The listing builds one solid part. Answer for the finished solid, in the listing's coordinates (mm). Face numbers are marked on the shaded views. A direction names the side the tool comes from. Coordinates: 2 decimals unless noted, no trailing zeros. Loops run counter-clockwise (first coordinate to the right, second up) from the corner with the lowest first, then second, coordinate; pieces in that order, holes last. Notation, with made-up numbers: (67, -7) - (82, -7) arc R20 cw to (82, 18) - close; hole circle Ø7 at (73, 69). An arc over 180 degrees is marked (long way). Write each question's results on one line, items separated by ' | '. Start each with the question number.
(1) Find section A-A on z = -37.5. Determine the outline of the cut face in (x, y).
(2) Given pin 1 Ø6 at (x, z) = (44, -5) entering from +Y; pin 2 Ø10 at (x, y) = (135.5, 79) entering from +Z; pin 3 Ø12 at (x, z) = (49.5, -67) entering from +Y; pin 4 Ø10 at (x, z) = (126, -11.5) entering from -Y, each flat-ended and moving along its own axis, determine where each tip first touches the part or whether it passes through.
(3) For the marked faces 4, 5, 6 and 7, determine the directions among +Z, -Z, +X, -X, +Y, -Y from which every point of the face is accessible in a straight line to the end or side of a thin tool.
(4) Find section C-C on y = 20. Determine the outline of the cut face in (x, z), then the cut area to 4 significant figures.
(5) Find section B-B on x = -175. Determine the outline of the cut face in (y, z).
(6) Find section D-D on z = -17.5. Determine the outline of the cut face in (x, y), then the cut area to 3 significant figures.
(7) Determine the mould class of the marked faces 1, 2 and 3 for opening direction X: released by +X, released by -X, zero draft, split by the parting line, or undercut.
(8) Consider line 1 (X direction, y = 36, z = -46.5); line 2 (Y direction, x = 0, z = -19); line 3 (Y direction, x = 0, z = -1.9). Determine where each line is inside the solid, lowest interval first. Write a range as from..to.
from build123d import *

# Parameters (mm, degrees)
SUPPORT_BODY_DEPTH           = 75
RIB_FRONT_DEPTH              = 12.5
RIB_START                    = -12.5
RIB_BACK_DEPTH               = 12.5
MOUNTING_HOLES_SKETCH_R      = 12.5
MOUNTING_HOLES_2X_25_DEPTH   = 108.5
FLANGE_FILLET_R12_5_A_R      = 12.5
FLANGE_FILLET_R12_5_B_R      = 12.5
FLANGE_FILLET_R12_5_C_R      = 12.5
FLANGE_FILLET_R12_5_D_R      = 12.5
COUNTERBORE_FRONT_SKETCH_R   = 25
COUNTERBORE_FRONT_50X5_DEPTH = 5
SHAFT_BORE_SKETCH_R          = 20
SHAFT_BORE_40_DEPTH          = 98
COUNTERBORE_START            = -5
COUNTERBORE_BACK_SKETCH_R    = 25
COUNTERBORE_BACK_50X5_DEPTH  = 5


with BuildPart() as part:
    # Support Profile Sketch → Support Body (new body)
    with BuildSketch(Plane.XY):
        with BuildLine():
            Line((33.541019662, 30), (62.5, 30))
            Line((62.5, 30), (137.5, 105))
            Line((137.5, 105), (212.5, 105))
            Line((212.5, 105), (212.5, 90))
            Line((212.5, 90), (137.5, 90))
            Line((137.5, 90), (82.5, 30))
            Line((82.5, 30), (82.5, 0))
            Line((82.5, 0), (82.5, -30))
            Line((82.5, -30), (-82.5, -30))
            Line((-82.5, -30), (-82.5, 30))
            Line((-82.5, 30), (-137.5, 90))
            Line((-137.5, 90), (-212.5, 90))
            Line((-212.5, 90), (-212.5, 105))
            Line((-212.5, 105), (-137.5, 105))
            Line((-137.5, 105), (-62.5, 30))
            Line((-62.5, 30), (-33.541019662, 30))
            ThreePointArc((-33.541019662, 30), (0, 55), (33.541019662, 30))
        make_face()
    extrude(amount=-SUPPORT_BODY_DEPTH)

    # Rib Front Sketch → Rib Front (add)
    with BuildSketch(Plane.XY.offset(-12.5)):
        with BuildLine():
            Line((137.5, 105), (0, 55))
            ThreePointArc((0, 55), (20.916500663, 48.062430401), (33.541019662, 30))
            Line((33.541019662, 30), (62.5, 30))
            Line((62.5, 30), (137.5, 105))
        make_face()
        with BuildLine():
            ThreePointArc((-33.541019662, 30), (-20.916500663, 48.062430401), (0, 55))
            Line((0, 55), (-137.5, 105))
            Line((-137.5, 105), (-62.5, 30))
            Line((-62.5, 30), (-33.541019662, 30))
        make_face()
    extrude(amount=-RIB_FRONT_DEPTH)

    # Rib Back Sketch → Rib Back (add)
    with BuildSketch(Plane(origin=(0, 0, -62.5), x_dir=(-1, 0, 0), z_dir=(0, 0, -1)).offset(RIB_START)):
        with BuildLine():
            Line((137.5, 105), (0, 55))
            ThreePointArc((0, 55), (20.916500663, 48.062430401), (33.541019662, 30))
            Line((33.541019662, 30), (62.5, 30))
            Line((62.5, 30), (137.5, 105))
        make_face()
        with BuildLine():
            Line((0, 55), (-137.5, 105))
            Line((-137.5, 105), (-62.5, 30))
            Line((-62.5, 30), (-33.541019662, 30))
            ThreePointArc((-33.541019662, 30), (-20.916500663, 48.062430401), (0, 55))
        make_face()
    extrude(amount=RIB_BACK_DEPTH)

    # Mounting Holes Sketch → Mounting Holes 2xØ25 (cut)
    with BuildSketch(Plane(origin=(0, 105, 0), x_dir=(1, 0, 0), z_dir=(0, 1, 0))):
        with Locations(Location((175, 37.5, 0), (0, 0, 270))):
            Circle(MOUNTING_HOLES_SKETCH_R)
        with Locations(Location((-175, 37.5, 0), (0, 0, 90))):
            Circle(MOUNTING_HOLES_SKETCH_R)
    extrude(amount=-MOUNTING_HOLES_2X_25_DEPTH, mode=Mode.SUBTRACT)

    # Flange Fillet R12.5 A
    flange_fillet_r12_5_a_edges = [part.edges().sort_by_distance(p)[0] for p in [
        (212.5, 97.5, 0),
    ]]
    fillet(flange_fillet_r12_5_a_edges, radius=FLANGE_FILLET_R12_5_A_R)

    # Flange Fillet R12.5 B
    flange_fillet_r12_5_b_edges = [part.edges().sort_by_distance(p)[0] for p in [
        (212.5, 97.5, -75),
    ]]
    fillet(flange_fillet_r12_5_b_edges, radius=FLANGE_FILLET_R12_5_B_R)

    # Flange Fillet R12.5 C
    flange_fillet_r12_5_c_edges = [part.edges().sort_by_distance(p)[0] for p in [
        (-212.5, 97.5, -75),
    ]]
    fillet(flange_fillet_r12_5_c_edges, radius=FLANGE_FILLET_R12_5_C_R)

    # Flange Fillet R12.5 D
    flange_fillet_r12_5_d_edges = [part.edges().sort_by_distance(p)[0] for p in [
        (-212.5, 97.5, 0),
    ]]
    fillet(flange_fillet_r12_5_d_edges, radius=FLANGE_FILLET_R12_5_D_R)

    # Counterbore Front Sketch → Counterbore Front Ø50x5 (cut)
    with BuildSketch(Plane.XY):
        with Locations((0, 20)):
            Circle(COUNTERBORE_FRONT_SKETCH_R)
    extrude(amount=-COUNTERBORE_FRONT_50X5_DEPTH, mode=Mode.SUBTRACT)

    # Shaft Bore Sketch → Shaft Bore Ø40 (cut)
    with BuildSketch(Plane.XY.offset(-5)):
        with Locations((0, 20)):
            Circle(SHAFT_BORE_SKETCH_R)
    extrude(amount=-SHAFT_BORE_40_DEPTH, mode=Mode.SUBTRACT)

    # Counterbore Back Sketch → Counterbore Back Ø50x5 (cut)
    with BuildSketch(Plane(origin=(0, 0, -75), x_dir=(-1, 0, 0), z_dir=(0, 0, -1)).offset(COUNTERBORE_START)):
        with Locations(Location((0, 20, 0), (0, 0, 180))):
            Circle(COUNTERBORE_BACK_SKETCH_R)
    extrude(amount=COUNTERBORE_BACK_50X5_DEPTH, mode=Mode.SUBTRACT)


solid = part.part
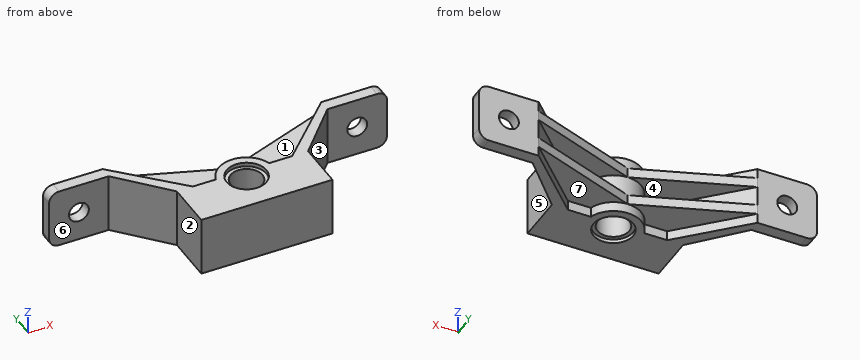
Values:
1) outline: (-212.5, 90) - (-187.5, 90) - (-187.5, 105) - (-212.5, 105) - close; (-162.5, 90) - (-137.5, 90) - (-82.5, 30) - (-82.5, -30) - (82.5, -30) - (82.5, 30) - (137.5, 90) - (162.5, 90) - (162.5, 105) - (137.5, 105) - (62.5, 30) - (33.54, 30) arc R35 ccw to (-33.54, 30) - (-62.5, 30) - (-137.5, 105) - (-162.5, 105) - close; (187.5, 90) - (212.5, 90) - (212.5, 105) - (187.5, 105) - close; hole circle Ø40 at (0, 20)
2) pin 1: stops at y = 30 | pin 2: passes through | pin 3: stops at y = 74.44 | pin 4: stops at y = 72
3) face 4: +Y | face 5: +Z, -Z, +X, -Y | face 6: +Z, -Z, -X, -Y | face 7: -Z, +Y
4) outline: (-82.5, -75) - (-25, -75) - (-25, -70) - (-20, -70) - (-20, -5) - (-25, -5) - (-25, 0) - (-82.5, 0) - close; (20, -70) - (25, -70) - (25, -75) - (82.5, -75) - (82.5, 0) - (25, 0) - (25, -5) - (20, -5) - close | area: 9,275 mm²
5) outline: (90, -75) - (105, -75) - (105, -50) - (90, -50) - close; (90, -25) - (105, -25) - (105, 0) - (90, 0) - close
6) outline: (-212.5, 90) - (-137.5, 90) - (-82.5, 30) - (-82.5, -30) - (82.5, -30) - (82.5, 30) - (137.5, 90) - (212.5, 90) - (212.5, 105) - (137.5, 105) - (0, 55) - (-137.5, 105) - (-212.5, 105) - close; hole circle Ø40 at (0, 20) | area: 21,300 mm²
7) face 1: undercut | face 2: released by -X | face 3: released by +X
8) line 1: x = -88..-68.5, -31.13..-12, 12..31.13, 68.5..88 | line 2: y = -30..0, 40..55 | line 3: y = -30..-5, 45..55
